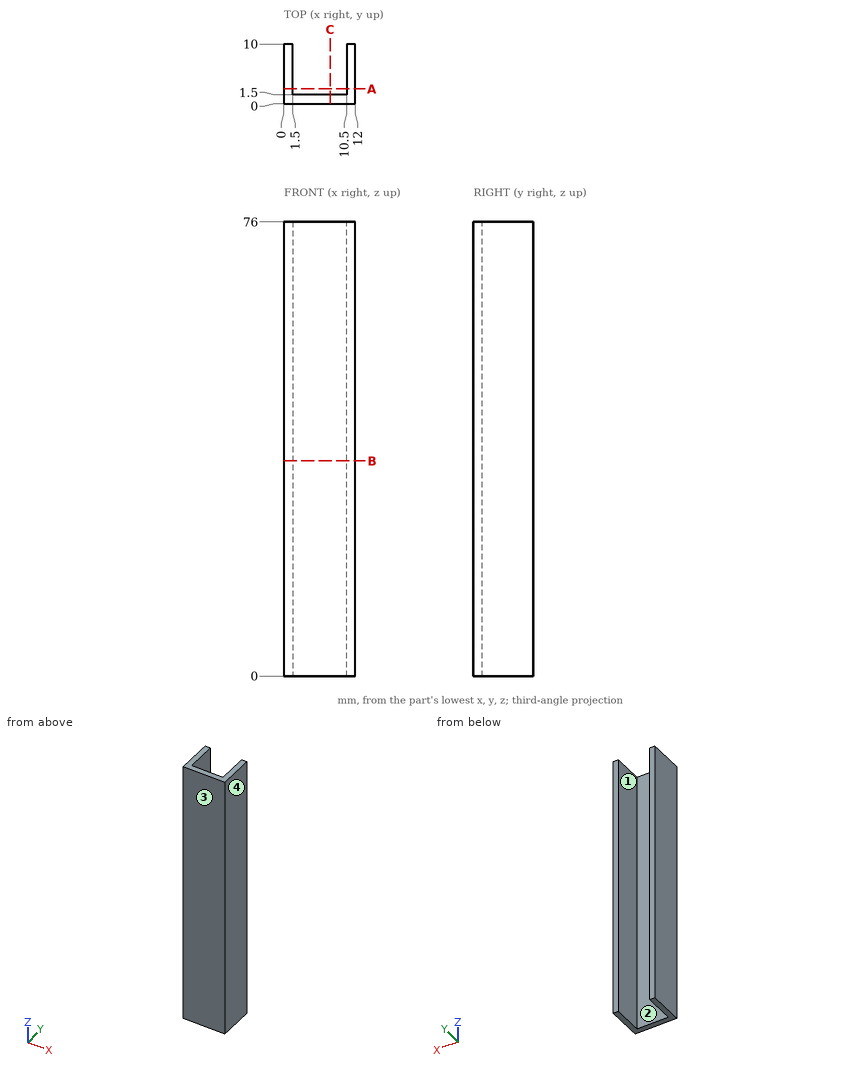
Input: dimensioned drawing with shaded views. Units: mm. Origin: part minimum x, y, z. Give positions to 0.01 mm unless a question says otherwise; leave off trailing zeros. Write each loop counter-clockwise with the first axis right and the second up, starting at its lowest first coordinate (ties: lowest second). Pieces come first, ordered by that corner, then holes.
Q1. Material intervals for probe 1 along X at (y, z) = (3.75, 67.5); probe 2 along Y at (x, z) = (4.5, 11), sorted ascending.
Q2. Section A-A, the plane y = 2.5. Output: boundary loops of the cut face in (x, z).
Q3. Section B-B, the plane z = 36. Output: boundary loops of the cut face in (x, y).
Q4. Pull-direction query (X, two-part tool) for the marked faces 1, 2, 3 and 4; classes: pulls with the +X half, pulls with the -X half, needs draft (parallel to the pull), parting line crosses it, or undercut.
Q5. Section C-C, the plane x = 7.75. Output: boundary loops of the cut face in (y, z).
Q6. First-contact query: P1, Ø4.5, axis at x = 6, z = 20.5, coming from the +Y side; P2, Ø2, axis at x = 9, y = 7, coming from the +Z side. Flat tips, straight axial feed; report the tip coordinate or a pass-through.
Filled in:
1. probe 1: x = 0 to 1.5, 10.5 to 12
1. probe 2: y = 0 to 1.5
2. outline: (0, 0) - (1.5, 0) - (1.5, 76) - (0, 76) - close; (10.5, 0) - (12, 0) - (12, 76) - (10.5, 76) - close
3. outline: (0, 0) - (12, 0) - (12, 10) - (10.5, 10) - (10.5, 1.5) - (1.5, 1.5) - (1.5, 10) - (0, 10) - close
4. face 1: undercut
4. face 2: undercut
4. face 3: needs draft
4. face 4: pulls with the +X half
5. outline: (0, 0) - (1.5, 0) - (1.5, 76) - (0, 76) - close
6. P1: stops at y = 1.5
6. P2: passes through
